Design review of the part built by this model. Coordinates are the model's own, in mm. A direction names the side the tool comes from. Coordinates: 2 decimals unless noted, no trailing zeros. Write each loop counter-clockwise with the first axis right and the second up, starting at its lowest first coordinate (ties: lowest second). Pieces come first, ordered by that corner, then holes.
Q1. Take a section at A-A (y = 0). Give the boundary of the cut face in (x, z), and give its area (3 significant figures).
Q2. Machinability: for faces 1 (the conical face through (-11.512, -19.863, 1.379)), 2 (the flat face through (8.234, 21.458, 1.749)), 3 (the cylindrical face through (-5.21, -19.31, 0.49)), which of the approach directions +Z, -Z, +X, -X, +Y, -Y give a long, thin tool a straight path to every point of the face, cutting with its end or side? Answer none if there is none.
Q3. Insertion check: pin 1 (1.7 mm diameter, centred on y = -12.5, z = 2.5, fed in from -X); pin 2 (3 mm diameter, centred on x = -15, y = -16.5, fed in from -Z); pin 3 (2 mm diameter, centred on x = -15, y = -20, fed in from -Z); pin 4 (1.5 mm diameter, centred on x = -5, z = 1.5, fed in from +Y). Each pin has a flat end and moves straight along its axis. Give the tip position at first contact, or say it passes through.
Q4. Mouldability with a two-part tool opening along X and no side actions: class faces 4 (the flat face through (-13.51, -18.6, 1.75)), 5 (the conical face through (22.19, 5.9, 1.38)), 6 (the cylindrical face through (10.034, 17.301, 0.493)), 7 (the flat face through (-2.4, -12.6, 1.9)) as pulls with the +X half, pulls with the -X half, needs draft (parallel to the pull), parting line crosses it, or undercut.
Q5. Take a section at C-C (z = 1.7). Give the boundary of the cut face in (x, y), and give its area (3 significant figures).
Q6. Take a section at B-B (x = 0). Give the boundary of the cut face in (y, z).
Q7. For probe 1 along X at (y, z) = (0, 0.3); probe 2 along X at (y, z) = (-8, 0.75); probe 3 along Y at (x, z) = (0, 0.4), list the stretches that pass through material, from the lowest coordinate up.
```python
from build123d import *

# Parameters (mm, degrees)
SKETCH3_OUTSIDE_W   = 68.728
SKETCH3_OUTSIDE_H   = 68.728
CUT_EXTRUDE2_DEPTH  = 3.797865
SKETCH4_W           = 4.8
SKETCH4_H           = 1
BOSS_EXTRUDE1_DEPTH = 5


with BuildPart() as part:
    # Sketch2 → Base-Revolve (revolve)
    with BuildSketch(Plane(origin=(0, 0, 0), x_dir=(0, 0, -1), z_dir=(1, 0, 0))):
        Polygon((-2.797845949, 26), (0, 20), (0, 0), (-1, 0), (-1, 20), (-3.797845949, 26), align=None)
    revolve(axis=Axis((0, 0, 0), (0, 0, 1)))

    # Sketch3 outside → Cut-Extrude2 (cut)
    # profile 1 of 2: a face of its own
    with BuildSketch(Plane.XY):
        Rectangle(SKETCH3_OUTSIDE_W, SKETCH3_OUTSIDE_H)
        with BuildLine():
            Line((-2.4, -19.855477834), (-2.4, -25.8889938))
            Line((-2.4, -25.8889938), (2.4, -25.8889938))
            Line((2.4, -25.8889938), (2.4, -19.855477834))
            ThreePointArc((2.4, -19.855477834), (15.867066806, -12.17522858), (19.800084541, 2.82075383))
            Line((19.800084541, 2.82075383), (25.628013437, 4.382342671))
            Line((25.628013437, 4.382342671), (24.38568202, 9.018786637))
            Line((24.38568202, 9.018786637), (18.557753125, 7.457197796))
            ThreePointArc((18.557753125, 7.457197796), (17.320508076, 10), (15.736999295, 12.342886745))
            Line((15.736999295, 12.342886745), (20.003339349, 16.6092268))
            Line((20.003339349, 16.6092268), (16.6092268, 20.003339349))
            Line((16.6092268, 20.003339349), (12.342886745, 15.736999295))
            ThreePointArc((12.342886745, 15.736999295), (10, 17.320508076), (7.457197796, 18.557753125))
            Line((7.457197796, 18.557753125), (9.018786637, 24.38568202))
            Line((9.018786637, 24.38568202), (4.382342671, 25.628013437))
            Line((4.382342671, 25.628013437), (2.82075383, 19.800084541))
            ThreePointArc((2.82075383, 19.800084541), (-15.867066806, 12.17522858), (-18.395348208, -7.849277948))
            Line((-18.395348208, -7.849277948), (-23.62052631, -10.866035931))
            Line((-23.62052631, -10.866035931), (-21.22052631, -15.022957869))
            Line((-21.22052631, -15.022957869), (-15.995348208, -12.006199886))
            ThreePointArc((-15.995348208, -12.006199886), (-14.142135624, -14.142135624), (-12.006199886, -15.995348208))
            Line((-12.006199886, -15.995348208), (-15.022957869, -21.22052631))
            Line((-15.022957869, -21.22052631), (-10.866035931, -23.62052631))
            Line((-10.866035931, -23.62052631), (-7.849277948, -18.395348208))
            ThreePointArc((-7.849277948, -18.395348208), (-5.176380902, -19.318516526), (-2.4, -19.855477834))
        make_face(mode=Mode.SUBTRACT)
    # profile 2 of 2: a face of its own
    with BuildSketch(Plane.XY):
        with BuildLine():
            Line((2.4, -15.059963479), (2.4, -11.75))
            Line((2.4, -11.75), (-2.4, -11.75))
            Line((-2.4, -11.75), (-2.4, -15.059963479))
            ThreePointArc((-2.4, -15.059963479), (0, 15.25), (2.4, -15.059963479))
        make_face()
    extrude(amount=CUT_EXTRUDE2_DEPTH, mode=Mode.SUBTRACT)

    # Sketch4 → Boss-Extrude1 (add)
    with BuildSketch(Plane.XY):
        with Locations((0, -12.25)):
            Rectangle(SKETCH4_W, SKETCH4_H)
    extrude(amount=BOSS_EXTRUDE1_DEPTH)


solid = part.part
```
Response:
1. outline: (-20, 0) - (-15.25, 0) - (-15.25, 1) - (-20, 1) - close; (15.25, 0) - (20, 0) - (20, 1) - (15.25, 1) - close
1. area: 9.50 mm2
2. face 1: -Z, -X, -Y
2. face 2: +Z, -Z, +X
2. face 3: +Z, -Z, -Y
3. pin 1: stops at x = -23.14
3. pin 2: passes through
3. pin 3: stops at z = 1.93
3. pin 4: stops at y = 19.5
4. face 4: pulls with the -X half
4. face 5: pulls with the +X half
4. face 6: undercut
4. face 7: undercut
5. outline: (-21.57, -9.68) arc R23.65 ccw to (-19.17, -13.84) - (-17.3, -12.76) arc R21.5 cw to (-19.7, -8.6) - close; (-13.84, -19.17) arc R23.65 ccw to (-9.68, -21.57) - (-8.6, -19.7) arc R21.5 cw to (-12.76, -17.3) - close; (-2.4, -23.52) arc R23.65 ccw to (2.4, -23.52) - (2.4, -21.37) arc R21.5 cw to (-2.4, -21.37) - close; (-2.4, -12.75) - (2.4, -12.75) - (2.4, -11.75) - (-2.4, -11.75) - close; (3.21, 21.26) arc R21.5 cw to (7.85, 20.02) - (8.41, 22.1) arc R23.65 ccw to (3.77, 23.34) - close; (13.41, 16.81) arc R21.5 cw to (16.81, 13.41) - (18.33, 14.94) arc R23.65 ccw to (14.94, 18.33) - close; (20.02, 7.85) arc R21.5 cw to (21.26, 3.21) - (23.34, 3.77) arc R23.65 ccw to (22.1, 8.41) - close
5. area: 66.7 mm2
6. outline: (-25.89, 2.75) - (-20, 0) - (-11.75, 0) - (-11.75, 5) - (-12.75, 5) - (-12.75, 1) - (-20, 1) - (-25.89, 3.75) - close; (15.25, 0) - (20, 0) - (20, 1) - (15.25, 1) - close
7. probe 1: x = -20 to -15.25, 15.25 to 20
7. probe 2: x = -18.66 to -12.98, 12.98 to 18.33
7. probe 3: y = -20.86 to -11.75, 15.25 to 20
